Geometry: final body of the model. Coordinates: model frame, mm. A direction names the side the tool comes from. Give positions to 0.01 mm unless a question says otherwise; leave off trailing zeros. Loops run counter-clockwise (first coordinate to the right, second up) from the corner with the lowest first, then second, coordinate; pieces in that order, holes last. Notation, with made-up numbers: M 48,28.25 L 105,28.25 A26 cw 105,63.25 Z; hole C 68.25,70 d6. An arc over 180 degrees is marked long. Put each result on its own line as item: value.
```python
from build123d import *

# Parameters (mm, degrees)
LINK_PROFILE_SKETCH_R = 5
LINK_PLATE_5MM_DEPTH  = 5


with BuildPart() as part:
    # Link Profile Sketch → Link Plate 5mm (new body)
    with BuildSketch(Plane(origin=(0, 0, 0), x_dir=(1, 0, 0), z_dir=(0, 1, 0))):
        with BuildLine():
            Line((-45, 10), (45, 10))
            ThreePointArc((45, 10), (55, 0), (45, -10))
            Line((45, -10), (-45, -10))
            ThreePointArc((-45, -10), (-55, 0), (-45, 10))
        make_face()
        with Locations(Location((-45, 0, 0), (0, 0, 270))):
            Circle(LINK_PROFILE_SKETCH_R, mode=Mode.SUBTRACT)
        with Locations(Location((45, 0, 0), (0, 0, 270))):
            Circle(LINK_PROFILE_SKETCH_R, mode=Mode.SUBTRACT)
        with BuildLine():
            Line((-25, 5), (25, 5))
            ThreePointArc((25, 5), (30, 0), (25, -5))
            Line((25, -5), (-25, -5))
            ThreePointArc((-25, -5), (-30, 0), (-25, 5))
        make_face(mode=Mode.SUBTRACT)
    extrude(amount=LINK_PLATE_5MM_DEPTH)


solid = part.part
```
Item 1: Section A-A on x = 14. Output: boundary loops of the cut face in (y, z), then the cut area to 3 significant figures.
Output values:
outline: M 0,-10 L 5,-10 L 5,-5 L 0,-5 Z; M 0,5 L 5,5 L 5,10 L 0,10 Z
area: 50.0 mm²
Item 2: Set-up query: faces 1 (the flat face through (1, 5, 7)), 2 (the cylindrical face through (-30, 2, 0)). Return all of +Z, -Z, +X, -X, +Y, -Y with unobstructed straight access to the full face (end or side cutting, diameter ignored); none if empty.
Output values:
face 1: +Z, -Z, +X, -X, +Y
face 2: +Y, -Y
Item 3: Line query: probe 1 along X at (y, z) = (1.3, 0); probe 2 along Z at (x, y) = (-25, 2.75); probe 3 along X at (y, z) = (1.3, -2.25). Output: solid intervals per line, ascending. Write a range as [from, to].
Output values:
probe 1: [-55, -50], [-40, -30], [30, 40], [50, 55]
probe 2: [-10, -5], [5, 10]
probe 3: [-54.74, -49.47], [-40.53, -29.47], [29.47, 40.53], [49.47, 54.74]
Item 4: Section B-B on z = 0. Output: boundary loops of the cut face in (x, y).
Output values:
outline: M -55,0 L -50,0 L -50,5 L -55,5 Z; M -40,0 L -30,0 L -30,5 L -40,5 Z; M 30,0 L 40,0 L 40,5 L 30,5 Z; M 50,0 L 55,0 L 55,5 L 50,5 Z
Item 5: Mould query, pull axis X, two halves, no side actions, for faces 3 (the cylindrical face through (30, 2, 0)), 4 (the cylindrical face through (55, 2, 0)), 5 (the flat face through (1, 0, 7)), 6 (the flat face through (0, 2, 5)). Classes: pulls with the +X half, pulls with the -X half, needs draft (parallel to the pull), parting line crosses it, or undercut.
Output values:
face 3: undercut
face 4: pulls with the +X half
face 5: needs draft
face 6: undercut
Item 6: Pin query (flat end, axial travel): pin 1 Ø1 at (y, z) = (3.5, 4.5) entering from +X. Return the tip coordinate at first contact, or that it passes through.
Output values:
pin 1: x = 54.17
Item 7: Section C-C on y = 2.9. Output: boundary loops of the cut face in (x, z).
Output values:
outline: M -45,-10 L 45,-10 A10 ccw 45,10 L -45,10 A10 ccw Z; hole C -45,0 d10; hole M -25,-5 L 25,-5 A5 ccw 25,5 L -25,5 A5 ccw Z; hole C 45,0 d10
